The model under review builds one solid part; all positions refer to its coordinate system, in mm. Face numbers are marked on the shaded views. Coordinates: 2 decimals unless noted, no trailing zeros. Write each loop counter-clockwise with the first axis right and the second up, starting at its lowest first coordinate (ties: lowest second). Pieces come first, ordered by that corner, then holes. Notation, with made-up numbers: (20, -38) - (71, -38) arc R31 cw to (71, 1) - close; hole circle Ø6 at (55, 78.5). An arc over 180 degrees is marked (long way). Answer as CSV lines item,"result". Start each with the question number.
```python
from build123d import *

# Parameters (mm, degrees)
SKETCH1_W            = 227
SKETCH1_H            = 217
BOSS_EXTRUDE1_DEPTH  = 1.2
SKETCH21_W           = 229.4
SKETCH21_H           = 219.4
SKETCH21_W_2         = 227
SKETCH21_H_2         = 217
BOSS_EXTRUDE2_DEPTH  = 30
SKETCH22_W           = 261
SKETCH22_H           = 235
SKETCH22_W_2         = 227
SKETCH22_H_2         = 217
BOSS_EXTRUDE3_DEPTH  = 1.2
SKETCH23_W           = 261
SKETCH23_H           = 30
CUT_EXTRUDE1_DEPTH   = 9
CUT_EXTRUDE2_START   = -28.8
SKETCH24_R           = 15
SKETCH24_R_2         = 60
CUT_EXTRUDE2_DEPTH   = 28.8
FILLET1_R            = 2
FILLET2_R            = 2
M4_CLEARANCE_HOLE1_D = 4.8


with BuildPart() as part:
    # Sketch1 → Boss-Extrude1 (new body)
    with BuildSketch(Plane.XY):
        Rectangle(SKETCH1_W, SKETCH1_H)
    extrude(amount=BOSS_EXTRUDE1_DEPTH)

    # Sketch21 → Boss-Extrude2 (add)
    with BuildSketch(Plane.XY.offset(1.2)):
        Rectangle(SKETCH21_W, SKETCH21_H)
        Rectangle(SKETCH21_W_2, SKETCH21_H_2, mode=Mode.SUBTRACT)
    extrude(amount=-BOSS_EXTRUDE2_DEPTH)

    # Sketch22 → Boss-Extrude3 (add)
    with BuildSketch(Plane(origin=(0, 0, -28.8), x_dir=(-1, 0, 0), z_dir=(0, 0, -1))):
        Rectangle(SKETCH22_W, SKETCH22_H)
        Rectangle(SKETCH22_W_2, SKETCH22_H_2, mode=Mode.SUBTRACT)
    extrude(amount=-BOSS_EXTRUDE3_DEPTH)

    # Sketch23 → Cut-Extrude1 (cut)
    with BuildSketch(Plane(origin=(0, 117.5, 0), x_dir=(1, 0, 0), z_dir=(0, 1, 0))):
        with Locations((0, 13.8)):
            Rectangle(SKETCH23_W, SKETCH23_H)
    extrude(amount=-CUT_EXTRUDE1_DEPTH, mode=Mode.SUBTRACT)

    # Sketch24 → Cut-Extrude2 (cut)
    with BuildSketch(Plane.XY.offset(1.2).offset(CUT_EXTRUDE2_START)):
        Circle(SKETCH24_R)
        with Locations((0, 135)):
            Circle(SKETCH24_R_2)
        with BuildLine():
            Line((-80, -40), (-80, 40))
            ThreePointArc((-80, 40), (-65, 55), (-50, 40))
            Line((-50, 40), (-50, -40))
            ThreePointArc((-50, -40), (-65, -55), (-80, -40))
        make_face()
        with BuildLine():
            Line((80, -40), (80, 40))
            ThreePointArc((80, 40), (65, 55), (50, 40))
            Line((50, 40), (50, -40))
            ThreePointArc((50, -40), (65, -55), (80, -40))
        make_face()
        with BuildLine():
            Line((10, -60), (10, -120))
            ThreePointArc((10, -120), (0, -130), (-10, -120))
            Line((-10, -120), (-10, -60))
            ThreePointArc((-10, -60), (0, -50), (10, -60))
        make_face()
    extrude(amount=CUT_EXTRUDE2_DEPTH, mode=Mode.SUBTRACT)

    # Fillet1
    fillet1_edges = [part.edges().sort_by_distance(p)[0] for p in [
        (114.7, -0.6, 1.2),
        (-113.5, 0, 0),
        (113.5, 0, 0),
        (-114.7, -0.6, 1.2),
    ]]
    fillet(fillet1_edges, radius=FILLET1_R)

    # Fillet2
    fillet2_edges = [part.edges().sort_by_distance(p)[0] for p in [
        (-130.5, -117.5, -28.2),
        (130.5, -117.5, -28.2),
        (130.5, 108.5, -28.2),
        (-130.5, 108.5, -28.2),
    ]]
    fillet(fillet2_edges, radius=FILLET2_R)

    # M4 Clearance Hole1 (through all)
    with Locations(Plane.XY.offset(-27.6)):
        with Locations((-122.5, 80)):
            m4_clearance_hole1 = Hole(M4_CLEARANCE_HOLE1_D / 2)

    # Sketch pattern1: M4 Clearance Hole1 at 5 more places
    with Locations((0, -80, 0), (0, -160, 0), (245, -160, 0), (245, -80, 0), (245, 0, 0)):
        add(m4_clearance_hole1, mode=Mode.SUBTRACT)


solid = part.part
```
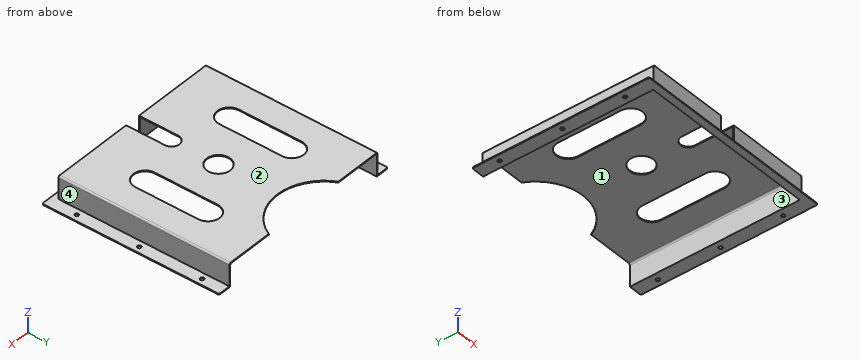
(1) Add section D-D on x = -93. Give the boundary of the cut face in (y, z), then the cut area to 3 significant figures.
(2) Add section C-C on x = -65. Give the boundary of the cut face in (y, z), then the cut area to 3 significant figures.
(3) Add section B-B on z = -7.5. Give the boundary of the cut face in (x, y).
(4) The part is to be moulded in two halves that separate along X. For the marked faces 1, 2, 3 and 4, say which applies: released by +X, released by -X, zero draft, split by the parting line, or undercut.
(5) Wall thickness on line 1 (Y direction, x = 122.5, z = -28.15); line 2 (X direction, y = 25.5, z = -20); line 3 (Y direction, x = -85, z = -4): over which ranges is each line inside the solid? List them lowest first.
(6) Add section A-A on y = -103.5. Give the boundary of the cut face in (x, z).
(7) For pin 1 (1.5 mm diameter, centred on x = 75.5, z = -18, fed in from +Y); pin 2 (3 mm diameter, centred on y = 0, z = -20, fed in from -X); pin 3 (8 mm diameter, centred on y = 24, z = -15, fed in from +X); pin 4 (3 mm diameter, centred on x = 122.5, y = -80, fed in from -Z), all flat-tipped, find the tip position at first contact; note any pin that passes through.
Reported:
1,outline,"(-117.5, -28.8) - (-108.5, -28.8) - (-108.5, 0) - (108.5, 0) - (108.5, 1.2) - (-109.7, 1.2) - (-109.7, -27.6) - (-117.5, -27.6) - close"
1,area,"306 mm²"
2,outline,"(-117.5, -28.8) - (-108.5, -28.8) - (-108.5, 0) - (-55, 0) - (-55, 1.2) - (-109.7, 1.2) - (-109.7, -27.6) - (-117.5, -27.6) - close; (55, 0) - (108.5, 0) - (108.5, 1.2) - (55, 1.2) - close"
2,area,"174 mm²"
3,outline,"(-114.7, -109.7) - (-10, -109.7) - (-10, -108.5) - (-113.5, -108.5) - (-113.5, 108.5) - (-114.7, 108.5) - close; (10, -109.7) - (114.7, -109.7) - (114.7, 108.5) - (113.5, 108.5) - (113.5, -108.5) - (10, -108.5) - close"
4,face 1,"undercut"
4,face 2,"zero draft"
4,face 3,"undercut"
4,face 4,"released by +X"
5,line 1,"-117.5 to -82.4, -77.6 to -2.4, 2.4 to 77.6, 82.4 to 108.5"
5,line 2,"-114.7 to -113.5, 113.5 to 114.7"
5,line 3,"-109.7 to -108.5"
6,outline,"(-130.5, -28.8) - (-113.5, -28.8) - (-113.5, -2) arc R2 cw to (-111.5, 0) - (-10, 0) - (-10, 1.2) - (-112.7, 1.2) arc R2 ccw to (-114.7, -0.8) - (-114.7, -27.6) - (-130.5, -27.6) - close; (10, 0) - (111.5, 0) arc R2 cw to (113.5, -2) - (113.5, -28.8) - (130.5, -28.8) - (130.5, -27.6) - (114.7, -27.6) - (114.7, -0.8) arc R2 ccw to (112.7, 1.2) - (10, 1.2) - close"
7,pin 1,"y = -108.5"
7,pin 2,"x = -114.7"
7,pin 3,"x = 114.7"
7,pin 4,"through"
